Design review of the part built by this model. Coordinates are the model's own, in mm. Coordinates: 2 decimals unless noted, no trailing zeros. Write each loop counter-clockwise with the first axis right and the second up, starting at its lowest first coordinate (ties: lowest second). Pieces come first, ordered by that corner, then holes. Notation, with made-up numbers: (50, 87.5) - (94, 87.5) arc R26 cw to (94, 107.5) - close; hole circle Ø7 at (-38, -39.5). An arc over 180 degrees is marked (long way). One line per item, written item: value.
from build123d import *

# Parameters (mm, degrees)
SKETCH1_R                  = 142.5
SKETCH1_R_2                = 25
BOSS_EXTRUDE1_DEPTH        = 6
F_20_0_20_DIAMETER_HOLE1_D = 20
F_16_0_16_DIAMETER_HOLE1_D = 16


with BuildPart() as part:
    # Sketch1 → Boss-Extrude1 (new, symmetric)
    with BuildSketch(Plane(origin=(0, 0, 0), x_dir=(1, 0, 0), z_dir=(0, 1, 0))):
        with Locations(Location((0, 0, 0), (0, 0, 270))):
            Circle(SKETCH1_R)
        with Locations(Location((0, 0, 0), (0, 0, 270))):
            Circle(SKETCH1_R_2, mode=Mode.SUBTRACT)
    extrude(amount=BOSS_EXTRUDE1_DEPTH, both=True)

    # Ø20.0 (20) Diameter Hole1 (through all)
    with Locations(Plane(origin=(0, 6, 0), x_dir=(1, 0, 0), z_dir=(0, 1, 0))):
        with Locations((0, 55), (55, 0), (0, -55), (-55, 0)):
            Hole(F_20_0_20_DIAMETER_HOLE1_D / 2)

    # Ø16.0 (16) Diameter Hole1 (through all)
    with Locations(Plane(origin=(0, 6, 0), x_dir=(1, 0, 0), z_dir=(0, 1, 0))):
        with Locations((0, 116), (39.674336626, 109.004344011), (74.563362724, 88.861155402), (100.458946839, 58), (114.237699349, 20.143188609), (114.237699349, -20.143188609), (100.458946839, -58), (74.563362724, -88.861155402), (39.674336626, -109.004344011), (0, -116), (-39.674336626, -109.004344011), (-74.563362724, -88.861155402), (-100.458946839, -58), (-114.237699349, -20.143188609), (-114.237699349, 20.143188609), (-100.458946839, 58), (-74.563362724, 88.861155402), (-39.674336626, 109.004344011)):
            Hole(F_16_0_16_DIAMETER_HOLE1_D / 2)


solid = part.part
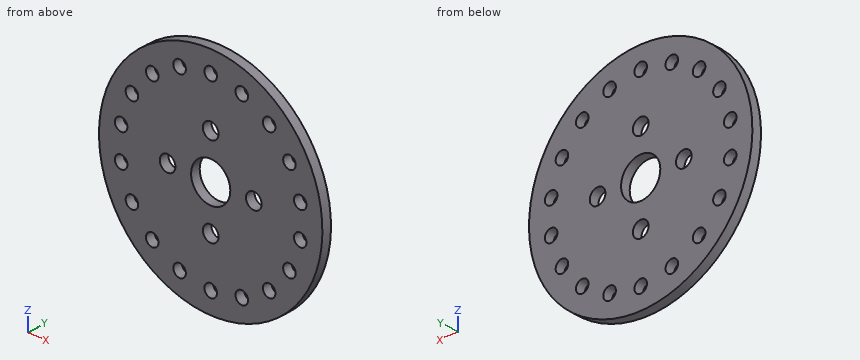
1. Consider section A-A, the plane x = 0. Write out the cut boundary in (y, z).
Answer block:
outline: (-6, -142.5) - (6, -142.5) - (6, -124) - (-6, -124) - close; (-6, -108) - (6, -108) - (6, -65) - (-6, -65) - close; (-6, -45) - (6, -45) - (6, -25) - (-6, -25) - close; (-6, 25) - (6, 25) - (6, 45) - (-6, 45) - close; (-6, 65) - (6, 65) - (6, 108) - (-6, 108) - close; (-6, 124) - (6, 124) - (6, 142.5) - (-6, 142.5) - close
2. Consider section C-C, the plane x = 55. Write out the cut boundary in (y, z), then the cut area to 4 significant figures.
Answer block:
outline: (-6, -131.46) - (6, -131.46) - (6, -10) - (-6, -10) - close; (-6, 10) - (6, 10) - (6, 131.46) - (-6, 131.46) - close
area: 2,915 mm^2
3. Insertion check: pin 1 Ø13 at (x, z) = (114.24, 20.14) entering from -Y (3 decimals); pin 2 Ø4 at (y, z) = (-3, -36) entering from +X; pin 3 Ø23 at (x, z) = (-55, 0) entering from -Y; pin 4 Ø3 at (y, z) = (3, -91.5) entering from +X. Each pin has a flat end and moves straight along its axis. Give the tip position at first contact, or say it passes through.
Answer block:
pin 1: passes through
pin 2: stops at x = 138.38
pin 3: stops at y = -6
pin 4: stops at x = 110.48
4. Wall thickness on line 1 along X through (y, z) = (-2.75, -116); line 2 along Z through (x, y) = (-37.5, -3.25); line 3 along X through (y, z) = (5.5, 17): over which ranges is each line inside the solid? List them lowest first.
Answer block:
line 1: x = -82.77 to -43.56, -35.79 to -8, 8 to 35.79, 43.56 to 82.77
line 2: z = -137.48 to -116.7, -101.31 to 101.31, 116.7 to 137.48
line 3: x = -141.48 to -121.59, -106.88 to -18.33, 18.33 to 106.88, 121.59 to 141.48
5. Consider section D-D, the plane y = -1. Give the number of separate pieces and of enclosed holes in the cut face, then the cut area to 3 significant figures.
Answer block:
separate pieces: 1
enclosed holes: 23
area: 57,000 mm^2
6. Consider section B-B, the plane z = 0. Write out the cut boundary in (x, y).
Answer block:
outline: (-142.5, -6) - (-65, -6) - (-65, 6) - (-142.5, 6) - close; (-45, -6) - (-25, -6) - (-25, 6) - (-45, 6) - close; (25, -6) - (45, -6) - (45, 6) - (25, 6) - close; (65, -6) - (142.5, -6) - (142.5, 6) - (65, 6) - close
